from build123d import *

# Parameters (mm, degrees)
BASE_STEP_BODY_DEPTH        = 80
UPPER_BLOCK_SKETCH_W        = 40
UPPER_BLOCK_SKETCH_H        = 20
UPPER_BLOCK_DEPTH           = 80
CORNER_NOTCH_SKETCH_25X25_W = 40
CORNER_NOTCH_SKETCH_25X25_H = 30
CORNER_NOTCH_25X25_DEPTH    = 20
SIDE_RECESS_DEPTH           = 183.277261336
SIDE_RECESS_DEPTH_BACK      = 20
SLOT_SKETCH_R               = 10
SLOT_CUT_DEPTH              = 40


with BuildPart() as part:
    # Base Step Profile Sketch → Base Step Body (new body)
    with BuildSketch(Plane.XY):
        Polygon((0, 0), (140, 0), (140, 80), (140, 85), (60, 85), (60, 35), (80, 35), (80, 20), (0, 20), align=None)
    extrude(amount=BASE_STEP_BODY_DEPTH)

    # Upper Block Sketch → Upper Block (add)
    with BuildSketch(Plane.XY.offset(80)):
        with Locations((120, 95)):
            Rectangle(UPPER_BLOCK_SKETCH_W, UPPER_BLOCK_SKETCH_H)
    extrude(amount=-UPPER_BLOCK_DEPTH)

    # Corner Notch Sketch 25x25 → Corner Notch 25x25 (cut)
    with BuildSketch(Plane(origin=(0, 105, 0), x_dir=(1, 0, 0), z_dir=(0, 1, 0))):
        with Locations((120, -40)):
            Rectangle(CORNER_NOTCH_SKETCH_25X25_W, CORNER_NOTCH_SKETCH_25X25_H)
    extrude(amount=-CORNER_NOTCH_25X25_DEPTH, mode=Mode.SUBTRACT)

    # Side Recess Sketch → Side Recess (cut, two sides: drawn at the far end of the back side and taken through both)
    with BuildSketch(Plane(origin=(0, 20, 0), x_dir=(1, 0, 0), z_dir=(0, 1, 0)).offset(-SIDE_RECESS_DEPTH_BACK)):
        Polygon((25, -30), (0, -15), (0, -65), (25, -50), (50, -50), (50, -40), (50, -30), align=None)
    extrude(amount=SIDE_RECESS_DEPTH + SIDE_RECESS_DEPTH_BACK, mode=Mode.SUBTRACT)

    # Slot Sketch → Slot Cut (cut)
    with BuildSketch(Plane.ZY.offset(-60)):
        with Locations((20, 60)):
            Circle(SLOT_SKETCH_R)
        with Locations((60, 60)):
            Circle(SLOT_SKETCH_R)
    extrude(amount=-SLOT_CUT_DEPTH, mode=Mode.SUBTRACT)


solid = part.part
Could you check a few things on this model? Use its own coordinates, in mm. A direction names the side the tool comes from. Round coordinates to 2 decimals unless told otherwise and drop trailing zeros. Write each loop counter-clockwise with the first axis right and the second up, starting at its lowest first coordinate (ties: lowest second). Pieces come first, ordered by that corner, then holes. Notation, with made-up numbers: (43.5, -11.75) - (49.5, -11.75) arc R29 ccw to (49.5, 22.25) - close; hole circle Ø9 at (61, 27). An arc over 180 degrees is marked (long way). Put each result on its own line as item: value. Start each with the question number.
(1) Will these pins go through, and if not, where does the flat tip stop? pin 1 (23 mm diameter, centred on y = 60, z = 60, fed in from -X); pin 2 (2 mm diameter, centred on x = 92, z = 25, fed in from -Y); pin 3 (8 mm diameter, centred on x = 93.5, z = 26, fed in from +Y); pin 4 (7.5 mm diameter, centred on y = 25.5, z = 25.5, fed in from -X).
(2) I want a section at C-C, the plane z = 12. Please give me the cut outline in (x, y), plus the area to 3 significant figures.
(3) Thinking about a two-plate mould opening in Y: for faces 1 (the flat face through (80, 28, 39)), 2 (the cylindrical face through (79.72, 56.17, 29.237)), 3 (the flat face through (85, 42, 0)), 4 (the flat face through (69, 0, 39)), which applies, released by +Y, released by -Y, zero draft, split by the parting line, or undercut?
(4) For faces 5 (the flat face through (60, 60, 39)), 6 (the cylindrical face through (80, 60, 50)), 7 (the flat face through (0, 10, 7)), 8 (the flat face through (12.325, 9.86, 57.605)), which set-ups out of +Z, -Z, +X, -X, +Y, -Y let a thin tool reach every point of the face, with its end or its side?
(5) I want a section at B-B, the plane y = 88.5. Please give me the cut outline in (x, z).
(6) I want a section at D-D, the plane x = 83. Please give me the cut outline in (y, z).
(7) I want a section at A-A, the plane x = 16.5. Please give me the cut outline in (y, z).
(8) I need wall thicknesses on probe 1 along Y at (x, z) = (72.5, 20); probe 2 along Y at (x, z) = (67, 63); probe 3 along Z at (x, y) = (72.5, 69). Which ranges of each line are inside material? Lowest first, please.
Here are the results:
1. pin 1: stops at x = 60
1. pin 2: stops at y = 0
1. pin 3: stops at y = 85
1. pin 4: stops at x = 80
2. outline: (0, 0) - (140, 0) - (140, 105) - (100, 105) - (100, 85) - (60, 85) - (60, 66) - (100, 66) - (100, 54) - (60, 54) - (60, 35) - (80, 35) - (80, 20) - (0, 20) - close
2. area: 8,020 mm^2
3. face 1: undercut
3. face 2: undercut
3. face 3: zero draft
3. face 4: released by -Y
4. face 5: +Z, -Z, -X, +Y
4. face 6: -X
4. face 7: +Z, -Z, -X, +Y, -Y
4. face 8: -X, +Y, -Y
5. outline: (100, 0) - (140, 0) - (140, 25) - (100, 25) - close; (100, 55) - (140, 55) - (140, 80) - (100, 80) - close
6. outline: (0, 0) - (85, 0) - (85, 80) - (0, 80) - close; hole circle Ø20 at (60, 20); hole circle Ø20 at (60, 60)
7. outline: (0, 0) - (20, 0) - (20, 24.9) - (0, 24.9) - close; (0, 55.1) - (20, 55.1) - (20, 80) - (0, 80) - close
8. probe 1: y = 0 to 20, 35 to 50, 70 to 85
8. probe 2: y = 0 to 20, 35 to 50.46, 69.54 to 85
8. probe 3: z = 0 to 15.64, 24.36 to 55.64, 64.36 to 80
